```python
from build123d import *

# Parameters (mm, degrees)
SKETCH_1_W                   = 100
SKETCH_1_H                   = 125
EXTRUDE_1_DEPTH              = 20
HOLE_WIZARD_M8_1_D           = 8.5
HOLE_WIZARD_M8_1_CBORE_D     = 15
HOLE_WIZARD_M8_1_CBORE_DEPTH = 8
SKETCH_4_R                   = 43
CUT_EXTRUDE_1_DEPTH          = 83.5
HOLE_WIZARD_M6_1_D           = 5
FILLET_1_R                   = 10


with BuildPart() as part:
    # 草图1 → 凸台-拉伸1 (new body)
    with BuildSketch(Plane.XY):
        Rectangle(SKETCH_1_W, SKETCH_1_H)
    extrude(amount=EXTRUDE_1_DEPTH)

    # M8 六角凹头螺钉的柱形沉头孔1 (through all)
    with Locations(Plane.XY.offset(20)):
        with Locations((-30, -52.5), (30, -52.5)):
            hole_wizard_m8_1 = CounterBoreHole(HOLE_WIZARD_M8_1_D / 2, HOLE_WIZARD_M8_1_CBORE_D / 2, HOLE_WIZARD_M8_1_CBORE_DEPTH)

    # 草图4 → 切除-拉伸1 (cut, through all)
    with BuildSketch(Plane.XY.offset(20)):
        Circle(SKETCH_4_R)
    extrude(amount=-CUT_EXTRUDE_1_DEPTH, mode=Mode.SUBTRACT)

    # M6 螺纹孔1 (through all)
    with Locations(Plane.XY.offset(20)):
        with Locations((-18.368804754, 44.346217561), (18.368804754, 44.346217561)):
            hole_wizard_m6_1 = Hole(HOLE_WIZARD_M6_1_D / 2)

    # 镜向2: M8 六角凹头螺钉的柱形沉头孔1, M6 螺纹孔1 across plane
    add(hole_wizard_m8_1.mirror(Plane.ZX), mode=Mode.SUBTRACT)
    add(hole_wizard_m6_1.mirror(Plane.ZX), mode=Mode.SUBTRACT)

    # 圆角1
    fillet_1_edges = [part.edges().sort_by_distance(p)[0] for p in [
        (-50, 62.5, 10),
        (50, 62.5, 10),
        (50, -62.5, 10),
        (-50, -62.5, 10),
    ]]
    fillet(fillet_1_edges, radius=FILLET_1_R)


solid = part.part
```
CAD build for the part. Positions are in the model's coordinates, mm. A direction names the side the tool comes from. Give positions to 0.01 mm unless a question says otherwise; leave off trailing zeros. Order: outer loops, then holes, each group sorted by start corner. A loop starts at its lowest first (then second) coordinate and runs counter-clockwise, first axis right, second up.
(1) Flat gauge pins, fed straight in: pin 1 (6 mm diameter, centred on x = -18.37, y = -44.35, fed in from -Z); pin 2 (7.5 mm diameter, centred on x = -28.5, y = 51, fed in from +Z); pin 3 (4 mm diameter, centred on x = 18.37, y = -44.35, fed in from -Z). Where does each tip first touch, or does it go through?
(2) Tool access for faces 4 (the cylindrical face through (24.5, 47.4, 16.1)), 5 (the cylindrical face through (-26.63, 55.09, 5.92)): list every direction of +Z, -Z, +X, -X, +Y, -Y with a clear straight run to the whole face (end or side of a thin tool).
(3) Saw through at D-D, the plane x = -30. Give the cut face in (y, z).
(4) Mould opens along X. For faces 1 (the cylindrical face through (46.99, -59.65, 10.14)), 2 (the flat face through (-12, 43, 20)), 3 (the cylindrical face through (17.215, 42.128, 9.86)) say: released by +X, released by -X, zero draft, split by the parting line, or undercut.
(5) Saw through at C-C, the plane z = 18.25. State how many separate pieces and enclosed holes the cut face has, then the cut area to 3 significant figures.
(6) Saw through at B-B, the plane y = 0. Give the cut face in (x, z), then the cut area to 3 significant figures.
(7) Saw through at A-A, the plane x = 0. Give the cut face in (y, z), then the cut area to 3 significant figures.
(8) Drill centre lines: L1, parallel to X at y = 52.5, z = 9.75; L2, parallel to Y at x = -1, z = 14; L3, parallel to X at y = 56, z = 2. Where is each one in solid material? Low to high.
Results found:
1. pin 1: stops at z = 0
1. pin 2: stops at z = 12
1. pin 3: passes through
2. face 4: +Z
2. face 5: +Z, -Z
3. outline: (-62.5, 0) - (-56.75, 0) - (-56.75, 12) - (-60, 12) - (-60, 20) - (-62.5, 20) - close; (-48.25, 0) - (-30.81, 0) - (-30.81, 20) - (-45, 20) - (-45, 12) - (-48.25, 12) - close; (30.81, 0) - (48.25, 0) - (48.25, 12) - (45, 12) - (45, 20) - (30.81, 20) - close; (56.75, 0) - (62.5, 0) - (62.5, 20) - (60, 20) - (60, 12) - (56.75, 12) - close
4. face 1: released by +X
4. face 2: zero draft
4. face 3: undercut
5. separate pieces: 1
5. enclosed holes: 9
5. area: 5,820 mm2
6. outline: (-50, 0) - (-43, 0) - (-43, 20) - (-50, 20) - close; (43, 0) - (50, 0) - (50, 20) - (43, 20) - close
6. area: 280 mm2
7. outline: (-62.5, 0) - (-43, 0) - (-43, 20) - (-62.5, 20) - close; (43, 0) - (62.5, 0) - (62.5, 20) - (43, 20) - close
7. area: 780 mm2
8. L1: x = -50 to -34.25, -25.75 to 25.75, 34.25 to 50
8. L2: y = -62.5 to -42.99, 42.99 to 62.5
8. L3: x = -49.37 to -32.41, -27.59 to 27.59, 32.41 to 49.37
